```python
from build123d import *

# Parameters (mm, degrees)
SKETCH1_W                                           = 240
SKETCH1_H                                           = 92
BOSS_EXTRUDE1_DEPTH                                 = 10
CUT_EXTRUDE1_DEPTH                                  = 10
SKETCH3_W                                           = 180
SKETCH3_H                                           = 49
CUT_EXTRUDE2_DEPTH                                  = 10
FILLET1_R                                           = 10
CHAMFER1_SIZE                                       = 3
M4_TAPPED_HOLE1_D                                   = 3.3
M4_TAPPED_HOLE1_DEPTH                               = 11.5
M4_TAPPED_HOLE1_TIP                                 = 0.991420021
CBORE_FOR_M6_HEX_SOCKET_HEAD_CAP_SCREW1_D           = 6.4
CBORE_FOR_M6_HEX_SOCKET_HEAD_CAP_SCREW1_CBORE_D     = 11
CBORE_FOR_M6_HEX_SOCKET_HEAD_CAP_SCREW1_CBORE_DEPTH = 6.4
SKETCH8_W                                           = 130
SKETCH8_H                                           = 89
CUT_EXTRUDE3_DEPTH                                  = 1


with BuildPart() as part:
    # Sketch1 → Boss-Extrude1 (new body)
    with BuildSketch(Plane.XY):
        Rectangle(SKETCH1_W, SKETCH1_H)
    extrude(amount=BOSS_EXTRUDE1_DEPTH)

    # Sketch2 → Cut-Extrude1 (cut)
    with BuildSketch(Plane.XY.offset(10)):
        with BuildLine():
            Line((-95, -21.7), (105, -21.7))
            ThreePointArc((105, -21.7), (108.3, -25), (105, -28.3))
            Line((105, -28.3), (-95, -28.3))
            ThreePointArc((-95, -28.3), (-98.3, -25), (-95, -21.7))
        make_face()
    extrude(amount=-CUT_EXTRUDE1_DEPTH, mode=Mode.SUBTRACT)

    # Sketch3 → Cut-Extrude2 (cut)
    with BuildSketch(Plane.XY.offset(10)):
        with Locations((-30, 21.5)):
            Rectangle(SKETCH3_W, SKETCH3_H)
    extrude(amount=-CUT_EXTRUDE2_DEPTH, mode=Mode.SUBTRACT)

    # Fillet1
    fillet1_edges = [part.edges().sort_by_distance(p)[0] for p in [
        (60, -3, 5),
    ]]
    fillet(fillet1_edges, radius=FILLET1_R)

    # Chamfer1
    chamfer1_edges = [part.edges().sort_by_distance(p)[0] for p in [
        (-120, -3, 5),
        (60, 46, 5),
        (120, -46, 5),
        (-120, -46, 5),
        (120, 46, 5),
    ]]
    chamfer(chamfer1_edges, length=CHAMFER1_SIZE)

    # M4 Tapped Hole1
    with Locations(Plane.XY.offset(10)):
        with Locations((-114, -17.5), (-114, -31.5)):
            Hole(M4_TAPPED_HOLE1_D / 2, depth=M4_TAPPED_HOLE1_DEPTH)
            with Locations((0, 0, -(M4_TAPPED_HOLE1_DEPTH + M4_TAPPED_HOLE1_TIP / 2))):  # 118° drill point
                Cone(0, M4_TAPPED_HOLE1_D / 2, M4_TAPPED_HOLE1_TIP, mode=Mode.SUBTRACT)

    # CBORE for M6 Hex Socket Head Cap Screw1 (through all)
    with Locations(Plane.XY.offset(10)):
        with Locations((67.5, 39), (112.5, 39)):
            CounterBoreHole(CBORE_FOR_M6_HEX_SOCKET_HEAD_CAP_SCREW1_D / 2, CBORE_FOR_M6_HEX_SOCKET_HEAD_CAP_SCREW1_CBORE_D / 2, CBORE_FOR_M6_HEX_SOCKET_HEAD_CAP_SCREW1_CBORE_DEPTH)

    # Sketch8 → Cut-Extrude3 (cut)
    with BuildSketch(Plane(origin=(0, 0, 0), x_dir=(-1, 0, 0), z_dir=(0, 0, -1))):
        with Locations((5, -1.5)):
            Rectangle(SKETCH8_W, SKETCH8_H)
    extrude(amount=-CUT_EXTRUDE3_DEPTH, mode=Mode.SUBTRACT)


solid = part.part
```
Model file for the job. Use its own axes, mm. A direction names the side the tool comes from. Give positions to 0.01 mm unless a question says otherwise; leave off trailing zeros. Write each loop counter-clockwise with the first axis right and the second up, starting at its lowest first coordinate (ties: lowest second). Pieces come first, ordered by that corner, then holes. Notation, with made-up numbers: (-18, 40.5) -> (14, 40.5) arc R11 ccw to (14, 54.5) -> close; hole circle Ø10 at (-3, -37.75). An arc over 180 degrees is marked (long way). Use CSV: the item, a comma, the result in double quotes. Start each with the question number.
1) Drill centre lines: L1, parallel to Y at x = 67.5, z = 7.25; L2, parallel to X at y = 34.5, z = 8.5; L3, parallel to X at y = 38.5, z = 4.25. Where is each one in solid material? Low to high.
2) Pin check, flat tips, straight feed: P1, Ø19.5, axis at x = 26, y = -39, coming from the -Z side; P2, Ø5, axis at x = -37, z = 4.5, coming from the +Y side; P3, Ø3, axis at x = -114, y = -17.5, coming from the +Z side. Stop position of each tip, or through.
3) Cut at B-B on x = -33. List the corners of the cut face in (y, z), plus the area to 3 significant figures.
4) Cut at C-C on z = 7. List the corners of the cut face in (x, y).
5) Two-plate mould, pull along Y, no slides. Class faces 1 (the flat face through (69.9, 36.6, 3.6)), 2 (the flat face through (120, -1, 5)), 3 (the flat face through (-35, -3, 5)): released by +Y, released by -Y, zero draft, split by the parting line, or undercut.
6) Tool access for faces 4 (the flat face through (-120, -25, 5)), 5 (the cylindrical face through (62, 39, 7)), 6 (the cylindrical face through (108.3, -24.9, 5.1)), 7 (the flat face through (-4, -10, 1)), 8 (the flat face through (-2, -46, 5)): list every direction of +Z, -Z, +X, -X, +Y, -Y with a clear straight run to the whole face (end or side of a thin tool).
7) Cut at D-D on x = 67.5. List the corners of the cut face in (y, z).
8) Cut at A-A on y = -25. List the corners of the cut face in (x, z), plus the area to 3 significant figures.
Final values:
1,L1,"y = -46 to -28.3, -21.7 to 33.5, 44.5 to 46"
1,L2,"x = 60 to 64.34, 70.66 to 109.34, 115.66 to 120"
1,L3,"x = 60 to 62.02, 72.98 to 107.02, 117.98 to 120"
2,P1,"stops at z = 1"
2,P2,"stops at y = -3"
2,P3,"passes through"
3,outline,"(-46, 1) -> (-28.3, 1) -> (-28.3, 10) -> (-46, 10) -> close; (-21.7, 1) -> (-3, 1) -> (-3, 10) -> (-21.7, 10) -> close"
3,area,"328 mm2"
4,outline,"(-120, -43) -> (-117, -46) -> (117, -46) -> (120, -43) -> (120, 43) -> (117, 46) -> (63, 46) -> (60, 43) -> (60, 7) arc R10 cw to (50, -3) -> (-117, -3) -> (-120, -6) -> close; hole circle Ø3.3 at (-114, -31.5); hole circle Ø3.3 at (-114, -17.5); hole (-95, -28.3) -> (105, -28.3) arc R3.3 ccw to (105, -21.7) -> (-95, -21.7) arc R3.3 ccw to start; hole circle Ø11 at (67.5, 39); hole circle Ø11 at (112.5, 39)"
5,face 1,"undercut"
5,face 2,"zero draft"
5,face 3,"released by +Y"
6,face 4,"+Z, -Z, -X, +Y, -Y"
6,face 5,"+Z"
6,face 6,"+Z, -Z"
6,face 7,"-Z, +Y, -Y"
6,face 8,"+Z, -Z, +X, -X, -Y"
7,outline,"(-46, 0) -> (-28.3, 0) -> (-28.3, 10) -> (-46, 10) -> close; (-21.7, 0) -> (35.8, 0) -> (35.8, 3.6) -> (33.5, 3.6) -> (33.5, 10) -> (-21.7, 10) -> close; (42.2, 0) -> (46, 0) -> (46, 10) -> (44.5, 10) -> (44.5, 3.6) -> (42.2, 3.6) -> close"
8,outline,"(-120, 0) -> (-98.3, 0) -> (-98.3, 10) -> (-120, 10) -> close; (108.3, 0) -> (120, 0) -> (120, 10) -> (108.3, 10) -> close"
8,area,"334 mm2"
